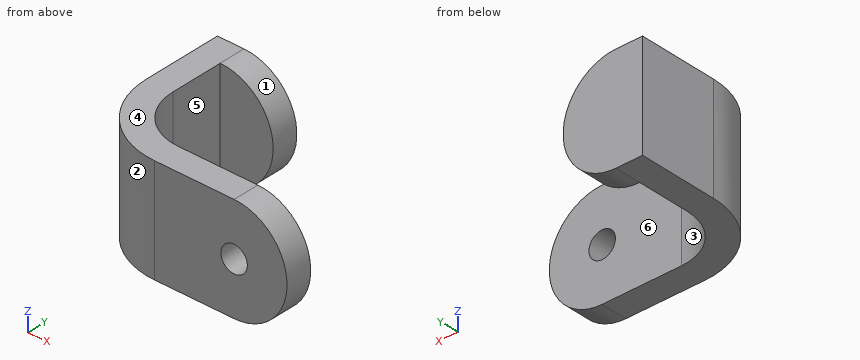
from build123d import *

# Parameters (mm, degrees)
CURVED_BRACKET_WALL_DEPTH = 40
ROUNDED_END_TAB_DEPTH     = 10
MOUNTING_TAB_DEPTH        = 10
MOUNTING_HOLE_SKETCH_R    = 5
MOUNTING_HOLE_10_DEPTH    = 10


with BuildPart() as part:
    # Bracket Profile Sketch → Curved Bracket Wall (new body)
    with BuildSketch(Plane.XY):
        with BuildLine():
            Line((50, 0), (20, 0))
            ThreePointArc((20, 0), (5.857864376, 5.857864376), (0, 20))
            Line((0, 20), (0, 50))
            Line((0, 50), (-10, 50))
            Line((-10, 50), (-10, 20))
            ThreePointArc((-10, 20), (-1.213203436, -1.213203436), (20, -10))
            Line((20, -10), (50, -10))
            Line((50, -10), (50, 0))
        make_face()
    extrude(amount=CURVED_BRACKET_WALL_DEPTH)

    # Rounded Tab Sketch → Rounded End Tab (add)
    with BuildSketch(Plane(origin=(0, 50, 0), x_dir=(1, 0, 0), z_dir=(0, 1, 0))):
        with BuildLine():
            Line((0, 0), (0, -40))
            ThreePointArc((0, -40), (20, -20), (0, 0))
        make_face()
    extrude(amount=-ROUNDED_END_TAB_DEPTH)

    # Mounting Tab Sketch → Mounting Tab (add)
    with BuildSketch(Plane(origin=(0, 0, 0), x_dir=(1, 0, 0), z_dir=(0, 1, 0))):
        with BuildLine():
            Line((50, 0), (50, -40))
            ThreePointArc((50, -40), (70, -20), (50, 0))
        make_face()
    extrude(amount=-MOUNTING_TAB_DEPTH)

    # Mounting Hole Sketch → Mounting Hole Ø10 (cut)
    with BuildSketch(Plane(origin=(0, 0, 0), x_dir=(1, 0, 0), z_dir=(0, 1, 0))):
        with Locations(Location((50, -20, 0), (0, 0, 270))):
            Circle(MOUNTING_HOLE_SKETCH_R)
    extrude(amount=-MOUNTING_HOLE_10_DEPTH, mode=Mode.SUBTRACT)


solid = part.part
Check sheet for the modelled part. Datum: model origin and axes. Units: mm. Face numbers are marked on the shaded views. A direction names the side the tool comes from. Give positions to 0.01 mm unless a question says otherwise; leave off trailing zeros. Loops run counter-clockwise (first coordinate to the right, second up) from the corner with the lowest first, then second, coordinate; pieces in that order, holes last. Notation, with made-up numbers: M -16,18.5 L 23,18.5 A9 cw 23,30.5 Z; hole C -8.5,48 d10. An arc over 180 degrees is marked long. Use a Markdown table: item, result. Add a question column.
Q1. Go/stop test with flat-tipped pins: pin 1 (16 mm diameter, centred on x = 50, z = 20, fed in from -Y); pin 2 (22 mm diameter, centred on x = 6.5, z = 12.5, fed in from -Y); pin 3 (3 mm diameter, centred on x = 35, y = 3, fed in from -Z); pin 4 (10 mm diameter, centred on y = 31.5, z = 28, fed in from +X). Record where each tip stops, or that it passes through.
Q2. Sectioned sample at C-C, the plane z = 6. Record the cut outline in (x, y).
Q3. Sectioned sample at A-A, the plane z = 20. Record the cut outline in (x, y).
Q4. Sectioned sample at B-B, the plane x = 12. Record the cut outline in (y, z).
Q5. Tool access check on the marked faces 1, 2 and 3. Record the directions out of +Z, -Z, +X, -X, +Y, -Y that give a thin tool (end or side, any length) a straight path to the whole face; none if there is none.
Q6. Scan lines: line 1 along Y through (x, z) = (15.5, 28); line 2 along X through (y, z) = (31, 20.5). Record each from-to range of solid material in increasing order. Write a range as [from, to].
Q7. Mould release check, pull along Y, two halves, no side actions. Record for the marked faces 4, 5 and 6: pulls with the +Y half, pulls with the -Y half, needs draft (parallel to the pull), parting line crosses it, or undercut.
Q8. Sectioned sample at D-D, the plane y = 29. Record the cut outline in (x, z), then the cut area to 3 significant figures.
Verdict:
| question | item | result |
|---|---|---|
| 1 | pin 1 | y = -10 |
| 1 | pin 2 | y = -9.9 |
| 1 | pin 3 | through |
| 1 | pin 4 | x = 0 |
| 2 | outline | M -10,20 A30 ccw 20,-10 L 64.28,-10 L 64.28,0 L 20,0 A20 cw 0,20 L 0,40 L 14.28,40 L 14.28,50 L -10,50 Z |
| 3 | outline | M -10,20 A30 ccw 20,-10 L 45,-10 L 45,0 L 20,0 A20 cw 0,20 L 0,40 L 20,40 L 20,50 L -10,50 Z; M 55,-10 L 70,-10 L 70,0 L 55,0 Z |
| 4 | outline | M -8.91,0 L 1.67,0 L 1.67,40 L -8.91,40 Z; M 40,4 L 50,4 L 50,36 L 40,36 Z |
| 5 | face 1 | +X, +Y |
| 5 | face 2 | +Z, -Z, -X, -Y |
| 5 | face 3 | +Z, -Z, +X |
| 6 | line 1 | [-9.66, 0.51], [40, 50] |
| 6 | line 2 | [-10, 0] |
| 7 | face 4 | needs draft |
| 7 | face 5 | undercut |
| 7 | face 6 | pulls with the +Y half |
| 8 | outline | M -10,0 L 0,0 L 0,40 L -10,40 Z |
| 8 | area | 400 mm^2 |
